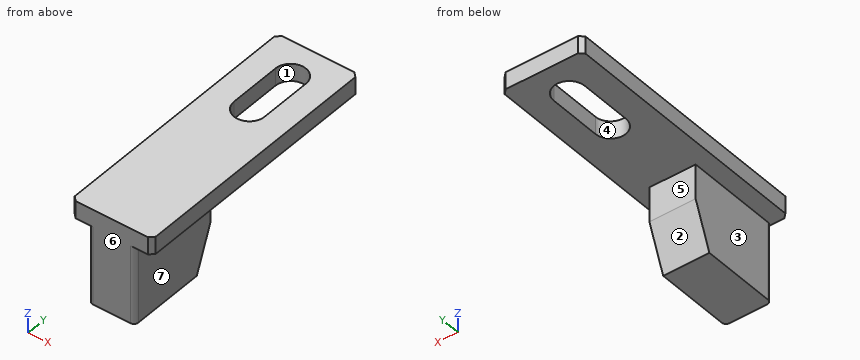
```python
from build123d import *

# Parameters (mm, degrees)
SKETCH1_W           = 5.3
SKETCH1_H           = 11
BOSS_EXTRUDE1_DEPTH = 9
SKETCH2_W           = 9.3
SKETCH2_H           = 30
BOSS_EXTRUDE2_DEPTH = 2
CUT_EXTRUDE1_DEPTH  = 10
CHAMFER1_SIZE       = 0.5
FILLET1_R           = 0.5
CHAMFER2_SIZE       = 2
CHAMFER2_SIZE2      = 5


with BuildPart() as part:
    # Sketch1 → Boss-Extrude1 (new body)
    with BuildSketch(Plane.XY):
        Rectangle(SKETCH1_W, SKETCH1_H)
    extrude(amount=BOSS_EXTRUDE1_DEPTH)

    # Sketch2 → Boss-Extrude2 (add)
    with BuildSketch(Plane.XY.offset(9)):
        with Locations((0, 9.5)):
            Rectangle(SKETCH2_W, SKETCH2_H)
    extrude(amount=BOSS_EXTRUDE2_DEPTH)

    # Sketch3 → Cut-Extrude1 (cut)
    with BuildSketch(Plane.XY.offset(11)):
        with BuildLine():
            Line((1.75, 20.5), (1.75, 14.5))
            ThreePointArc((1.75, 14.5), (0, 12.75), (-1.75, 14.5))
            Line((-1.75, 14.5), (-1.75, 20.5))
            ThreePointArc((-1.75, 20.5), (0, 22.25), (1.75, 20.5))
        make_face()
    extrude(amount=-CUT_EXTRUDE1_DEPTH, mode=Mode.SUBTRACT)

    # Chamfer1
    chamfer1_edges = [part.edges().sort_by_distance(p)[0] for p in [
        (-4.65, -5.5, 10),
        (4.65, -5.5, 10),
        (4.65, 24.5, 10),
        (-4.65, 24.5, 10),
    ]]
    chamfer(chamfer1_edges, length=CHAMFER1_SIZE)

    # Fillet1
    fillet1_edges = [part.edges().sort_by_distance(p)[0] for p in [
        (2.65, -5.5, 4.5),
        (-2.65, -5.5, 4.5),
    ]]
    fillet(fillet1_edges, radius=FILLET1_R)

    # Chamfer2
    chamfer2_edges = [part.edges().sort_by_distance(p)[0] for p in [
        (0, 5.5, 0),
    ]]
    chamfer2_side = [part.faces().sort_by_distance(p)[0] for p in [
        (0, 0.00993546, 0),
    ]]
    chamfer(chamfer2_edges, length=CHAMFER2_SIZE, length2=CHAMFER2_SIZE2, reference=chamfer2_side[0])


solid = part.part
```
Geometry check sheet. Reference: the model listing, model coordinates, mm. Face numbers are marked on the shaded views. A direction names the side the tool comes from. Coordinates: 2 decimals unless noted, no trailing zeros. Order: outer loops, then holes, each group sorted by start corner. A loop starts at its lowest first (then second) coordinate and runs counter-clockwise, first axis right, second up. Notation, with made-up numbers: (75.5, 1.25) - (107.5, 1.25) arc R21 cw to (107.5, 24.25) - close; hole circle Ø2 at (-27, -28.5). An arc over 180 degrees is marked (long way). Answer as a JSON object with one key per item and string values. Group by question number.
Item 1: Depth check by flat-ended pin: pin 1 Ø1.5 at (y, z) = (1, 4.5) entering from -X; pin 2 Ø4 at (y, z) = (19.5, 5.5) entering from +X; pin 3 Ø5 at (x, z) = (2.5, 3) entering from +Y; pin 4 Ø3 at (x, y) = (0.5, 7.5) entering from -Z. Enter the tip coordinate at first touch or a pass-through.
Item 2: Sectioned sample at C-C, the plane y = -1. Record the cut outline in (x, z), and give its area (3 significant figures).
Item 3: Sectioned sample at D-D, the plane y = 20. Record the cut outline in (x, z), and give its area (3 significant figures).
Item 4: Scan lines: probe 1 along Z at (x, y) = (4, 13); probe 2 along X at (y, z) = (-2, 4.5); probe 3 along Y at (x, z) = (1.5, 10.5). Record each from-to range of solid material in increasing order.
Item 5: Tool access check on the marked faces 5, 6 and 7. Record the directions out of +Z, -Z, +X, -X, +Y, -Y that give a thin tool (end or side, any length) a straight path to the whole face; none if there is none.
Item 6: Draft check along Y on the marked faces 1, 2, 3 and 4. Enter one of: +Y half, -Y half, draft (parallel to the pull), parting line (faces both ways), or undercut.
Item 7: Sectioned sample at B-B, the plane z = 9.5. Record the cut outline in (x, y), and give its area (3 significant figures).
Item 8: Sectioned sample at A-A, the plane x = 0. Record the cut outline in (y, z), and give its area (3 significant figures).
Resolved:
{
 "1": {"pin 1": "x = -2.65", "pin 2": "through", "pin 3": "y = 5.5", "pin 4": "z = 9"},
 "2": {"outline": "(-4.65, 9) - (-2.65, 9) - (-2.65, 0) - (2.65, 0) - (2.65, 9) - (4.65, 9) - (4.65, 11) - (-4.65, 11) - close", "area": "66.3 mm^2"},
 "3": {"outline": "(-4.65, 9) - (-1.75, 9) - (-1.75, 11) - (-4.65, 11) - close; (1.75, 9) - (4.65, 9) - (4.65, 11) - (1.75, 11) - close", "area": "11.6 mm^2"},
 "4": {"probe 1": "9 to 11", "probe 2": "-2.65 to 2.65", "probe 3": "-5.5 to 13.6, 21.4 to 24.5"},
 "5": {"face 5": "-Z, +X, -X, +Y", "face 6": "+Z, -Z, +X, -X, -Y", "face 7": "-Z, +X, +Y, -Y"},
 "6": {"face 1": "undercut", "face 2": "+Y half", "face 3": "draft", "face 4": "undercut"},
 "7": {"outline": "(-4.65, -5) - (-4.15, -5.5) - (4.15, -5.5) - (4.65, -5) - (4.65, 24) - (4.15, 24.5) - (-4.15, 24.5) - (-4.65, 24) - close; hole (-1.75, 14.5) arc R1.75 ccw to (1.75, 14.5) - (1.75, 20.5) arc R1.75 ccw to (-1.75, 20.5) - close", "area": "248 mm^2"},
 "8": {"outline": "(-5.5, 0) - (3.5, 0) - (5.5, 5) - (5.5, 9) - (12.75, 9) - (12.75, 11) - (-5.5, 11) - close; (22.25, 9) - (24.5, 9) - (24.5, 11) - (22.25, 11) - close", "area": "135 mm^2"}
}
